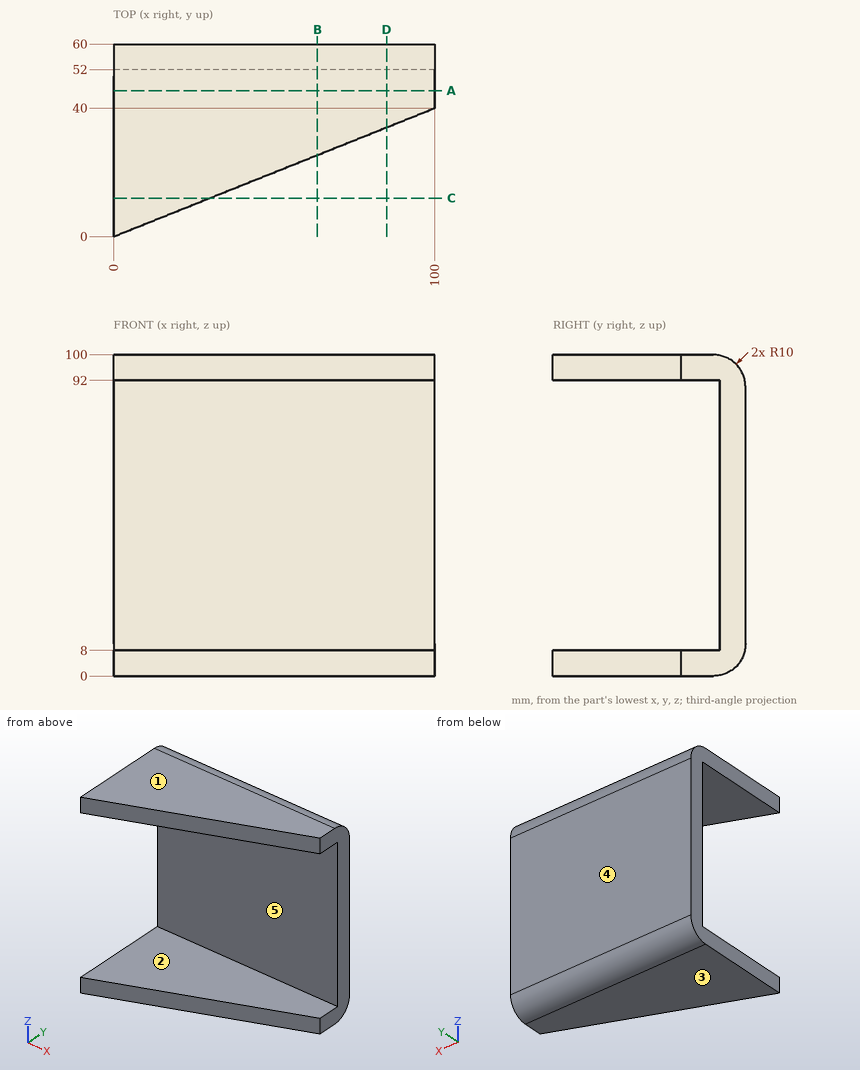
Geometry check sheet. Reference: drawing and pictorial views, mm from the part's lowest x, y, z. A direction names the side the tool comes from. Round coordinates to 2 decimals unless told otherwise and drop trailing zeros. Order: outer loops, then holes, each group sorted by start corner. A loop starts at its lowest first (then second) coordinate and runs counter-clockwise, first axis right, second up. Notation, with made-up numbers: M -8.75,32.25 L 24.25,32.25 A32 cw 24.25,69.25 Z; hole C 48,5.25 d9. An arc over 180 degrees is marked long. Answer as CSV lines item,"result".
1) Sectioned sample at A-A on y = 45.5. Record the cut outline in (x, z).
Entries:
outline,"M 0,0 L 100,0 L 100,8 L 0,8 Z; M 0,92 L 100,92 L 100,100 L 0,100 Z"
2) Gauge pin test, flat end, axial feed: pin 1 Ø2 at (x, z) = (50.5, 66) entering from -Y. Record the tip position at first contact, or that the pin passes through.
Entries:
pin 1,"y = 52"
3) Thickness scan on probe 1 along Z at (x, y) = (83, 48.5); probe 2 along Y at (x, z) = (83, 23); probe 3 along Z at (x, y) = (67, 53.5). Record the ranges inside material, lowest first. Write a range as [from, to].
Entries:
probe 1,"[0, 8], [92, 100]"
probe 2,"[52, 60]"
probe 3,"[0.63, 99.37]"
4) Sectioned sample at D-D on x = 85. Record the cut outline in (y, z), and give its area (3 significant figures).
Entries:
outline,"M 34,0 L 50,0 A10 ccw 60,10 L 60,90 A10 ccw 50,100 L 34,100 L 34,92 L 52,92 L 52,8 L 34,8 Z"
area,"1,050 mm2"
5) Mould release check, pull along Z, two halves, no side actions. Record for the marked faces 3, 4 and 5: +Z half, -Z half, draft (parallel to the pull), parting line (faces both ways), or undercut.
Entries:
face 3,"-Z half"
face 4,"draft"
face 5,"undercut"
6) Sectioned sample at B-B on x = 63.5. Record the cut outline in (y, z).
Entries:
outline,"M 25.4,0 L 50,0 A10 ccw 60,10 L 60,90 A10 ccw 50,100 L 25.4,100 L 25.4,92 L 52,92 L 52,8 L 25.4,8 Z"
7) Tool access check on the marked faces 1 and 2. Record the directions out of +Z, -Z, +X, -X, +Y, -Y that give a thin tool (end or side, any length) a straight path to the whole face; none if there is none.
Entries:
face 1,"+Z, +X, -X, +Y, -Y"
face 2,"+X, -X, -Y"
8) Sectioned sample at C-C on y = 12. Record the cut outline in (x, z).
Entries:
outline,"M 0,0 L 30,0 L 30,8 L 0,8 Z; M 0,92 L 30,92 L 30,100 L 0,100 Z"
